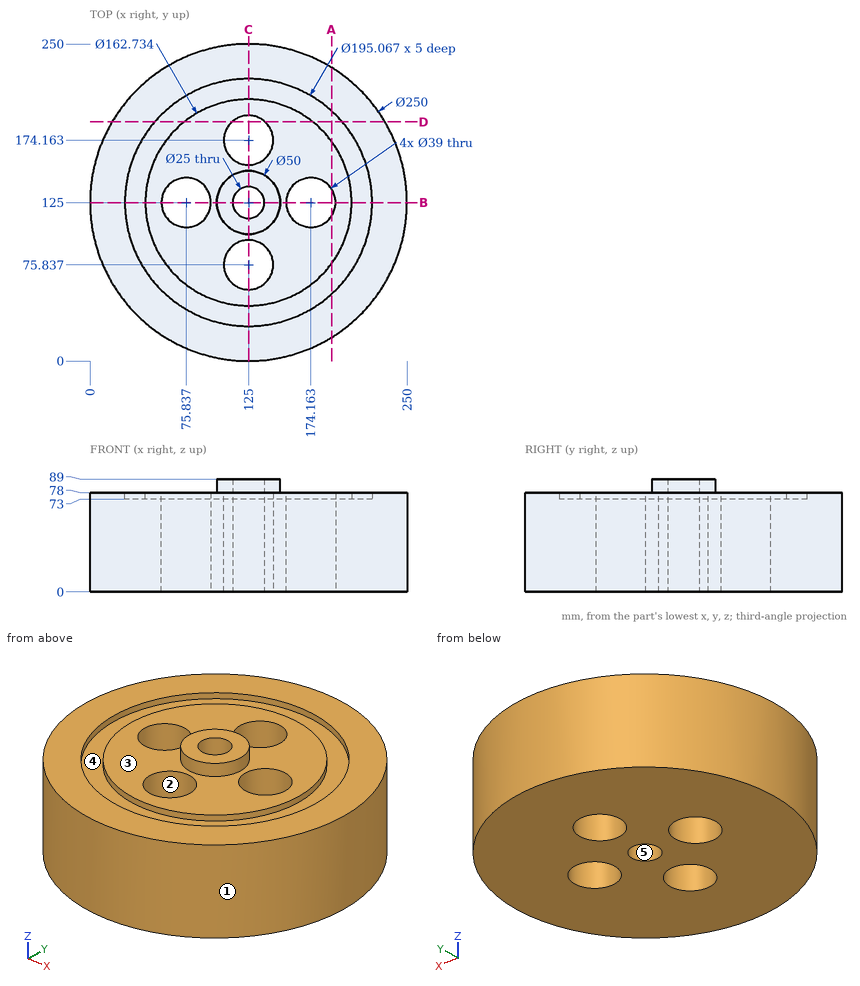
Here's the drawing with two shaded views (mm, measured from the low corner). I have some questions. A direction names the side the tool comes from. Coordinates: 2 decimals unless noted, no trailing zeros. Loops run counter-clockwise (first coordinate to the right, second up) from the corner with the lowest first, then second, coordinate; pieces in that order, holes last. Notation, with made-up numbers: (25, 18.25) -> (39, 18.25) arc R20 ccw to (39, 54.25) -> close; hole circle Ø3 at (-22.5, -7). An arc over 180 degrees is marked (long way). Use one line per item in the form item = value. Start each with the question number.
(1) Please list where these lines run through material, in increasing order: line 1 along Y through (x, z) = (125, 37.5); line 2 along Y through (x, z) = (125, 74); line 3 along Y through (x, z) = (111.5, 67) (1 decimal).
(2) We'd pull the mould along X, two halves only. Please class the marked faces 1, 2 and 3: pulls with the +X half, pulls with the -X half, needs draft (parallel to the pull), parting line crosses it, or undercut.
(3) If we section it at D-D (y = 188.5): Please give me the cut outline in (x, z), then the cut area to 3 significant figures.
(4) On a 3-axis mill with a long thin cutter (end or side, diameter ignored), from which of +Z, -Z, +X, -X, +Y, -Y can I reach the whole of each face in a straight line? I mean the marked faces 4 and 5. Say none if no direction works.
(5) If we section it at B-B (y = 125): Please give me the cut outline in (x, z), then the cut area to 3 significant figures.
(6) If we section it at A-A (x = 190.5): Please give me the cut outline in (y, z) (1 decimal).
(7) Will these pins go through, and if not, where does the flat tip stop? pin 1 (3 mm diameter, centred on y = 100.5, z = 53, fed in from +X); pin 2 (20 mm diameter, centred on x = 125, y = 125, fed in from +Z); pin 3 (10 mm diameter, centred on x = 197.5, y = 107.5, fed in from -Z); pin 4 (10 mm diameter, centred on x = 92.5, z = 11, fed in from -Y).
Verdict:
q1.line_1 = 0 to 56.34, 95.34 to 112.5, 137.5 to 154.66, 193.66 to 250
q1.line_2 = 0 to 27.47, 43.63 to 56.34, 95.34 to 112.5, 137.5 to 154.66, 193.66 to 206.37, 222.53 to 250
q1.line_3 = 0.7 to 61.8, 89.9 to 160.1, 188.2 to 249.3
q2.face_1 = parting line crosses it
q2.face_2 = undercut
q2.face_3 = needs draft
q3.outline = (17.33, 0) -> (111.78, 0) -> (111.78, 78) -> (74.12, 78) -> (74.12, 73) -> (50.97, 73) -> (50.97, 78) -> (17.33, 78) -> close; (138.22, 0) -> (232.67, 0) -> (232.67, 78) -> (199.03, 78) -> (199.03, 73) -> (175.88, 73) -> (175.88, 78) -> (138.22, 78) -> close
q3.area = 14,500 mm²
q4.face_4 = +Z
q4.face_5 = +Z, -Z
q5.outline = (0, 0) -> (56.34, 0) -> (56.34, 78) -> (43.63, 78) -> (43.63, 73) -> (27.47, 73) -> (27.47, 78) -> (0, 78) -> close; (95.34, 0) -> (112.5, 0) -> (112.5, 89) -> (100, 89) -> (100, 78) -> (95.34, 78) -> close; (137.5, 0) -> (154.66, 0) -> (154.66, 78) -> (150, 78) -> (150, 89) -> (137.5, 89) -> close; (193.66, 0) -> (250, 0) -> (250, 78) -> (222.53, 78) -> (222.53, 73) -> (206.37, 73) -> (206.37, 78) -> (193.66, 78) -> close
q5.area = 11,600 mm²
q6.outline = (18.5, 0) -> (114.4, 0) -> (114.4, 78) -> (76.7, 78) -> (76.7, 73) -> (52.7, 73) -> (52.7, 78) -> (18.5, 78) -> close; (135.6, 0) -> (231.5, 0) -> (231.5, 78) -> (197.3, 78) -> (197.3, 73) -> (173.3, 73) -> (173.3, 78) -> (135.6, 78) -> close
q7.pin_1 = 247.87
q7.pin_2 = through
q7.pin_3 = 0
q7.pin_4 = 3.06
